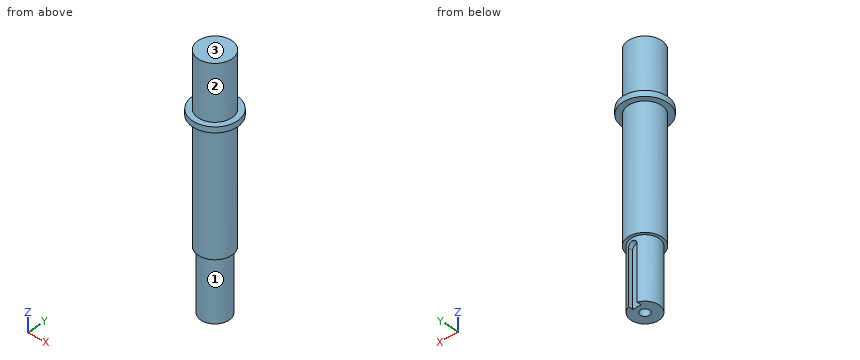
from build123d import *

# Parameters (mm, degrees)
SKETCH_1_R             = 6
EXTRUDE_1_DEPTH        = 65
SKETCH_2_R             = 5
EXTRUDE_2_DEPTH        = 22
SKETCH_3_W             = 2
SKETCH_3_H             = 2
ZJCQC_DEPTH            = 1.8
HOLE_WIZARD_M4_1_D     = 3.3
HOLE_WIZARD_M4_1_DEPTH = 10.1
HOLE_WIZARD_M4_1_TIP   = 0.991420021


with BuildPart() as part:
    # 草图1 → 凸台-拉伸1 (new body)
    with BuildSketch(Plane.XY):
        Circle(SKETCH_1_R)
    extrude(amount=EXTRUDE_1_DEPTH)

    # 草图2 → 凸台-拉伸2 (add)
    with BuildSketch(Plane(origin=(0, 0, 0), x_dir=(-1, 0, 0), z_dir=(0, 0, -1))):
        Circle(SKETCH_2_R)
    extrude(amount=EXTRUDE_2_DEPTH)

    # 草图3 → 旋转1 (revolve)
    with BuildSketch(Plane(origin=(0, 0, 0), x_dir=(1, 0, 0), z_dir=(0, 1, 0)), mode=Mode.PRIVATE) as revolve_1_sk:
        with Locations((-7, -44.5)):
            Rectangle(SKETCH_3_W, SKETCH_3_H)
    revolve(revolve_1_sk.sketch.rotate(Axis((0, 0, 65), (0, 0, -1)), 180), axis=Axis((0, 0, 65), (0, 0, -1)))

    # MyToolsZJC → ZJCQC (cut)
    with BuildSketch(Plane(origin=(0, 5, -22), x_dir=(0, 0, 1), z_dir=(0, 1, 0))):
        with BuildLine():
            Line((-0.5, 1.5), (19.5, 1.5))
            ThreePointArc((19.5, 1.5), (21, 0), (19.5, -1.5))
            Line((19.5, -1.5), (-0.5, -1.5))
            ThreePointArc((-0.5, -1.5), (-2, 0), (-0.5, 1.5))
        make_face()
    extrude(amount=-ZJCQC_DEPTH, mode=Mode.SUBTRACT)

    # M4 螺纹孔1
    with Locations(Plane(origin=(0, 0, -22), x_dir=(-1, 0, 0), z_dir=(0, 0, -1))):
        with Locations((0, 0)):
            Hole(HOLE_WIZARD_M4_1_D / 2, depth=HOLE_WIZARD_M4_1_DEPTH)
            with Locations((0, 0, -(HOLE_WIZARD_M4_1_DEPTH + HOLE_WIZARD_M4_1_TIP / 2))):  # 118° drill point
                Cone(0, HOLE_WIZARD_M4_1_D / 2, HOLE_WIZARD_M4_1_TIP, mode=Mode.SUBTRACT)


solid = part.part
Work out the finished part from the listing and answer in its coordinate system (mm). Face numbers are marked on the shaded views. A direction names the side the tool comes from. Give positions to 0.01 mm unless a question says otherwise; leave off trailing zeros. Write each loop counter-clockwise with the first axis right and the second up, starting at its lowest first coordinate (ties: lowest second). Pieces come first, ordered by that corner, then holes. Notation, with made-up numbers: M 71.5,10 L 101.5,10 A27 cw 101.5,46 Z; hole C 51.5,71 d9. An arc over 180 degrees is marked long. Answer as CSV lines item,"result".
Q1. Given P1, Ø5, axis at x = -0.5, z = 1.5, coming from the -Y side; P2, Ø8, axis at x = -2, z = -1, coming from the +Y side; P3, Ø1.3, axis at y = 4, z = -10.5, coming from the +X side, each flat-ended and moving along its own axis, determine where each tip first touches the part or whether it passes through.
A:
P1,"stops at y = -6"
P2,"stops at y = 6"
P3,"stops at x = 3.71"
Q2. A cutting plane is placed at A-A on z = 21. Write down the section's boundary in (x, y), plus the area to 3 significant figures.
A:
outline,"C 0,0 d12"
area,"113 mm²"
Q3. A tool of negligible diameter and unlimited length cuts with its end or side. For the marked faces 1, 2 and 3, from which of +Z, -Z, +X, -X, +Y, -Y can it reach the whole face along a straight path? Write none if from no direction.
A:
face 1,"-Z"
face 2,"+Z"
face 3,"+Z, +X, -X, +Y, -Y"
Q4. Find the intervals of material crossed by probe 1 along Y at (x, z) = (0, -18.75); probe 2 along X at (y, z) = (0, -17); probe 3 along Z at (x, y) = (-6, 4.25), in increasing order. Write a range as [from, to].
A:
probe 1,"y = [-5, -1.65], [1.65, 3.2]"
probe 2,"x = [-5, -1.65], [1.65, 5]"
probe 3,"z = [43.5, 45.5]"
